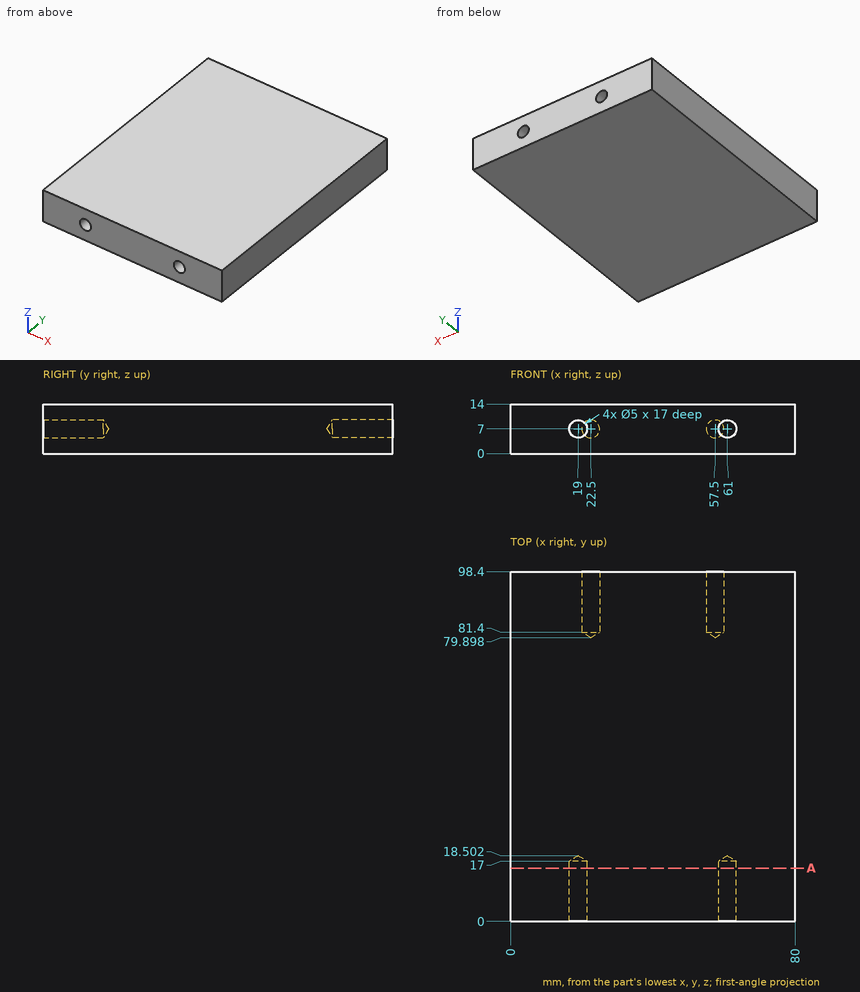
Geometry check sheet. Reference: drawing and pictorial views, mm from the part's lowest x, y, z. Give positions to 0.01 mm unless a question says otherwise; leave off trailing zeros. Order: outer loops, then holes, each group sorted by start corner. A loop starts at its lowest first (then second) coordinate and runs counter-clockwise, first axis right, second up. Notation, with made-up numbers: (-12, 4) - (-3, 4) arc R11 cw to (-3, 13) - close; hole circle Ø11 at (80, 64.5). An arc over 180 degrees is marked (long way). Use one line per item in the form item = value.
1) Sectioned sample at A-A (y = 15). Record the boundary of the cut face in (x, z).
Working result:
outline = (0, 0) - (80, 0) - (80, 14) - (0, 14) - close; hole circle Ø5 at (19, 7); hole circle Ø5 at (61, 7)
2) Depth check by flat-ended pin: pin 1 Ø3 at (x, z) = (19, 7) entering from -Y; pin 2 Ø4 at (x, z) = (22.5, 7) entering from +Y. Enter the tip coordinate at first touch or a pass-through.
Working result:
pin_1 = 17.6
pin_2 = 81.1
3) Material ranges on probe 1 along Z at (x, y) = (19, 8); probe 2 along X at (y, z) = (5, 5); probe 3 along Y at (x, z) = (17.5, 7), recorded low to high. Write a range as from..to.
Working result:
probe_1 = 0..4.5, 9.5..14
probe_2 = 0..17.5, 20.5..59.5, 62.5..80
probe_3 = 17.6..98.4
